Check sheet for the modelled part. Datum: model origin and axes. Units: mm. Face numbers are marked on the shaded views. A direction names the side the tool comes from. Round coordinates to 2 decimals unless told otherwise and drop trailing zeros. Write each loop counter-clockwise with the first axis right and the second up, starting at its lowest first coordinate (ties: lowest second). Pieces come first, ordered by that corner, then holes.
from build123d import *

# Parameters (mm, degrees)
OMEGA_PROFILE_SKETCH_R         = 14
OMEGA_BODY_DEPTH               = 28
SUPPORT_RIB_REACH              = 45.359
SUPPORT_RIB_SKETCH_WALL_W      = 114.016154836
SUPPORT_RIB_SKETCH_WALL_H      = 6
BASE_MOUNTING_HOLES_SKETCH_R   = 2
BASE_MOUNTING_HOLES_DEPTH      = 28
CLAMP_LUG_DEPTH                = 28
SPLIT_SLOT_SKETCH_W            = 2
SPLIT_SLOT_SKETCH_H            = 18.147677211
SPLIT_SLOT_2MM_DEPTH           = 28
CLAMP_SCREW_HOLES_SKETCH_R     = 2
CLAMP_SCREW_HOLES_3X_3_6_DEPTH = 28
EDGE_FILLETS_R0_8_R            = 0.8


with BuildPart() as part:
    # Omega Profile Sketch → Omega Body (new body)
    with BuildSketch(Plane.XY):
        with BuildLine():
            Line((-20, 0), (-20, -24))
            Line((-20, -24), (-28, -24))
            Line((-28, -24), (-28, -30))
            Line((-28, -30), (-15.6, -30))
            Line((-15.6, -30), (-15.6, -28.4))
            Line((-15.6, -28.4), (-14, -28.4))
            Line((-14, -28.4), (-14, -14.282856857))
            ThreePointArc((-14, -14.282856857), (0, -20), (14, -14.282856857))
            Line((14, -14.282856857), (14, -28.4))
            Line((14, -28.4), (15.6, -28.4))
            Line((15.6, -28.4), (15.6, -30))
            Line((15.6, -30), (28, -30))
            Line((28, -30), (28, -24))
            Line((28, -24), (20, -24))
            Line((20, -24), (20, 0))
            ThreePointArc((20, 0), (0, 20), (-20, 0))
        make_face()
        Circle(OMEGA_PROFILE_SKETCH_R, mode=Mode.SUBTRACT)
    extrude(amount=-OMEGA_BODY_DEPTH)

    # Support Rib Sketch wall → Support Rib (add, up to next)
    with BuildSketch(Plane(origin=(24, -12, -14), x_dir=(0.316227766017, -0.948683298051, 0), z_dir=(0.948683298051, 0.316227766017, 0)), mode=Mode.PRIVATE) as support_rib_sk1:
        Rectangle(SUPPORT_RIB_SKETCH_WALL_W, SUPPORT_RIB_SKETCH_WALL_H)
    support_rib_tool1 = extrude(support_rib_sk1.sketch, amount=-SUPPORT_RIB_REACH, mode=Mode.PRIVATE) - part.part
    support_rib = support_rib_tool1.solids().sort_by_distance((24, -12, -14))[0]
    add(support_rib)

    # Support Rib Mirror: Support Rib across plane
    add(support_rib.mirror(Plane(origin=(0, 0, 0), x_dir=(0, 0, 1), z_dir=(1, 0, 0))))

    # Base Mounting Holes Sketch → Base Mounting Holes (cut)
    with BuildSketch(Plane(origin=(0, -24, 0), x_dir=(1, 0, 0), z_dir=(0, 1, 0))):
        with Locations(Location((24, 22.5, 0), (0, 0, 270))):
            Circle(BASE_MOUNTING_HOLES_SKETCH_R)
        with Locations(Location((24, 5.5, 0), (0, 0, 270))):
            Circle(BASE_MOUNTING_HOLES_SKETCH_R)
        with Locations(Location((-24, 5.5, 0), (0, 0, 270))):
            Circle(BASE_MOUNTING_HOLES_SKETCH_R)
        with Locations(Location((-24, 22.5, 0), (0, 0, 270))):
            Circle(BASE_MOUNTING_HOLES_SKETCH_R)
    extrude(amount=-BASE_MOUNTING_HOLES_DEPTH, mode=Mode.SUBTRACT)

    # Clamp Lug Sketch → Clamp Lug (add)
    with BuildSketch(Plane.XY):
        with BuildLine():
            Line((-9, 17.860571099), (-9, 25.060571099))
            Line((-9, 25.060571099), (9, 25.060571099))
            Line((9, 25.060571099), (9, 17.860571099))
            ThreePointArc((9, 17.860571099), (0, 20), (-9, 17.860571099))
        make_face()
    extrude(amount=-CLAMP_LUG_DEPTH)

    # Split Slot Sketch → Split Slot 2mm (cut)
    with BuildSketch(Plane.XY):
        with Locations((0, 20.958575759)):
            Rectangle(SPLIT_SLOT_SKETCH_W, SPLIT_SLOT_SKETCH_H)
    extrude(amount=-SPLIT_SLOT_2MM_DEPTH, mode=Mode.SUBTRACT)

    # Clamp Screw Holes Sketch → Clamp Screw Holes 3xØ3.6 (cut)
    with BuildSketch(Plane(origin=(9, 0, 0), x_dir=(0, 0, -1), z_dir=(1, 0, 0))):
        with Locations(Location((6, 21.460571099, 0), (0, 0, 180))):
            Circle(CLAMP_SCREW_HOLES_SKETCH_R)
        with Locations(Location((14, 21.460571099, 0), (0, 0, 180))):
            Circle(CLAMP_SCREW_HOLES_SKETCH_R)
        with Locations(Location((22, 21.460571099, 0), (0, 0, 180))):
            Circle(CLAMP_SCREW_HOLES_SKETCH_R)
    extrude(amount=-CLAMP_SCREW_HOLES_3X_3_6_DEPTH, mode=Mode.SUBTRACT)

    # Edge Fillets R0.8
    edge_fillets_r0_8_edges = [part.edges().sort_by_distance(p)[0] for p in [
        (-20, -24, -5.5),
        (9, 17.860571099, -14),
        (-9, 17.860571099, -14),
        (5, 25.060571099, -28),
        (5, 25.060571099, 0),
        (-5, 25.060571099, 0),
        (-5, 25.060571099, -28),
        (20, -24, -22.5),
        (-20, -24, -22.5),
        (20, -24, -5.5),
    ]]
    fillet(edge_fillets_r0_8_edges, radius=EDGE_FILLETS_R0_8_R)


solid = part.part
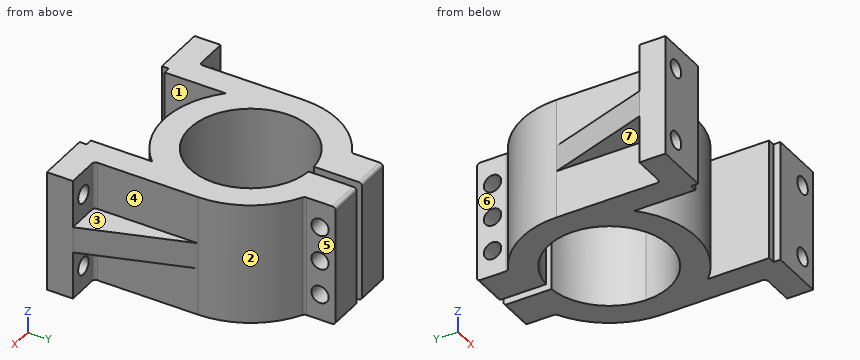
1. Scan lines: line 1 along Y through (x, z) = (7, -22) (3 decimals); line 2 along X through (y, z) = (21, -12); line 3 along X through (y, z) = (-18, -14.75). Record each from-to range of solid material in increasing order.
2. Go/stop test with flat-tipped pins: pin 1 (12 mm diameter, centred on y = -2.5, z = -25, fed in from -X); pin 2 (5 mm diameter, centred on x = 24, z = -22.5, fed in from +Y); pin 3 (3 mm diameter, centred on y = 16.5, z = -6.5, fed in from +X); pin 4 (10 mm diameter, centred on x = 21.5, y = -21, fed in from +Z). Record where each tip stops, or that it passes through.
3. Sectioned sample at D-D, the plane z = -18. Enter the section's corners in (x, y), plus the area to 3 significant figures.
4. Sectioned sample at A-A, the plane z = -14. Give the number of separate pieces and of enclosed holes in the cut face, plus the area to 3 significant figures.
5. Set-up check for the marked faces 4, 5, 6 and 7: record each of +Z, -Z, +X, -X, +Y, -Y from which the full face is reachable in a straight line by a thin tool's end or side.
6. Sectioned sample at B-B, the plane x = 5. Enter the section's corners in (y, z).
7. Sectioned sample at C-C, the plane y = 16. Enter the section's corners in (x, z), plus the area to 3 significant figures.
8. Release check for a two-part mould opening along X. For the marked faces 1, 2 and 3 record: released by +X, released by -X, zero draft, split by the parting line, or undercut.
Computed values:
1. line 1: y = -18.735 to -12.124, 12.124 to 19.461, 23.461 to 25.061
1. line 2: x = -9 to -1, 1 to 9
1. line 3: x = -26 to -14, -8.72 to 8.72, 14 to 26
2. pin 1: stops at x = -20
2. pin 2: stops at y = -24
2. pin 3: stops at x = 13.23
2. pin 4: stops at z = 0
3. outline: (-28, -30) - (-15.6, -30) - (-15.6, -28.4) - (-14, -28.4) - (-14, -14.28) arc R20 ccw to (14, -14.28) - (14, -28.4) - (15.6, -28.4) - (15.6, -30) - (28, -30) - (28, -24) - (20.8, -24) arc R0.8 cw to (20, -23.2) - (20, 0) arc R20 ccw to (9.42, 17.64) arc R0.8 cw to (9, 18.35) - (9, 25.06) - (1, 25.06) - (1, 13.96) arc R14 cw (long way) to (-1, 13.96) - (-1, 25.06) - (-9, 25.06) - (-9, 18.35) arc R0.8 cw to (-9.42, 17.64) arc R20 ccw to (-20, 0) - (-20, -23.2) arc R0.8 cw to (-20.8, -24) - (-28, -24) - close
3. area: 1,060 mm2
4. separate pieces: 3
4. enclosed holes: 0
4. area: 1,180 mm2
5. face 4: +Z, +X, +Y
5. face 5: +Z, -Z, +X, +Y
5. face 6: +Z, -Z, -X, +Y
5. face 7: -Z, -X, +Y
6. outline: (-19.36, -28) - (-13.08, -28) - (-13.08, 0) - (-19.36, 0) - close; (13.08, -28) - (24.26, -28) arc R0.8 ccw to (25.06, -27.2) - (25.06, -0.8) arc R0.8 ccw to (24.26, 0) - (13.08, 0) - close; hole circle Ø4 at (21.46, -22); hole circle Ø4 at (21.46, -14); hole circle Ø4 at (21.46, -6)
7. outline: (-12, -28) - (-1, -28) - (-1, 0) - (-12, 0) - close; (1, -28) - (12, -28) - (12, 0) - (1, 0) - close
7. area: 616 mm2
8. face 1: undercut
8. face 2: released by +X
8. face 3: zero draft
